Verification items for the finished model (mm, model axes). A direction names the side the tool comes from. Give positions to 0.01 mm unless a question says otherwise; leave off trailing zeros. Loops run counter-clockwise (first coordinate to the right, second up) from the corner with the lowest first, then second, coordinate; pieces in that order, holes last. Notation, with made-up numbers: M 36,28.25 L 46,28.25 A22 ccw 46,54.25 Z; hole C 35,87.5 d2. An arc over 180 degrees is marked long. Answer in a Markdown table with one row per item.
```python
from build123d import *

# Parameters (mm, degrees)
SKETCH1_W              = 10
SKETCH1_H              = 20
BOSS_EXTRUDE1_DEPTH    = 5
SKETCH2_W              = 10
SKETCH2_H              = 5
BOSS_EXTRUDE2_DEPTH    = 16
M2_5_CLEARANCE_HOLE1_D = 2.9
SKETCH6_W              = 10
SKETCH6_H              = 12
BOSS_EXTRUDE4_DEPTH    = 7
CHAMFER1_SIZE          = 3
CHAMFER1_SIZE2         = 5.196152423
FILLET1_R              = 4
CHAMFER2_SIZE          = 0.5
BOSS_EXTRUDE6_DEPTH    = 8
FILLET3_R              = 1
CHAMFER3_SIZE          = 0.5
CHAMFER3_SIZE2         = 2.83564091
SKETCH9_R              = 2
CUT_EXTRUDE1_DEPTH     = 2.1


with BuildPart() as part:
    # Sketch1 → Boss-Extrude1 (new body)
    with BuildSketch(Plane(origin=(0, 0, 0), x_dir=(1, 0, 0), z_dir=(0, 1, 0))):
        Rectangle(SKETCH1_W, SKETCH1_H)
    extrude(amount=BOSS_EXTRUDE1_DEPTH)

    # Sketch2 → Boss-Extrude2 (add)
    with BuildSketch(Plane(origin=(0, 0, 0), x_dir=(-1, 0, 0), z_dir=(0, -1, 0))):
        with Locations((0, 7.5)):
            Rectangle(SKETCH2_W, SKETCH2_H)
    extrude(amount=BOSS_EXTRUDE2_DEPTH)

    # M2.5 Clearance Hole1 (through all)
    with Locations(Plane.XY.offset(-5)):
        with Locations((0, -11.65), (0, -3.65)):
            Hole(M2_5_CLEARANCE_HOLE1_D / 2)

    # Sketch6 → Boss-Extrude4 (add)
    with BuildSketch(Plane.XY.offset(10)):
        with Locations((0, -1)):
            Rectangle(SKETCH6_W, SKETCH6_H)
    extrude(amount=BOSS_EXTRUDE4_DEPTH)

    # Chamfer1
    chamfer1_edges = [part.edges().sort_by_distance(p)[0] for p in [
        (0, 5, 17),
    ]]
    chamfer1_side = [part.faces().sort_by_distance(p)[0] for p in [
        (0, 5, 3.5),
    ]]
    chamfer(chamfer1_edges, length=CHAMFER1_SIZE, length2=CHAMFER1_SIZE2, reference=chamfer1_side[0])

    # Fillet1
    fillet1_edges = [part.edges().sort_by_distance(p)[0] for p in [
        (5, -7, 13.5),
        (-5, -7, 13.5),
    ]]
    fillet(fillet1_edges, radius=FILLET1_R)

    # Chamfer2
    chamfer2_edges = [part.edges().sort_by_distance(p)[0] for p in [
        (5, -16, -7.5),
        (-5, -16, -7.5),
    ]]
    chamfer(chamfer2_edges, length=CHAMFER2_SIZE)

    # Sketch8 → Boss-Extrude6 (add)
    with BuildSketch(Plane.XY.offset(17)):
        with BuildLine():
            ThreePointArc((-2.5, -4.5), (0, -7), (2.5, -4.5))
            ThreePointArc((2.5, -4.5), (0, -3.084524053), (-2.5, -4.5))
        make_face()
    extrude(amount=BOSS_EXTRUDE6_DEPTH)

    # Fillet3
    fillet3_edges = [part.edges().sort_by_distance(p)[0] for p in [
        (2.5, -4.5, 21),
        (-2.5, -4.5, 21),
    ]]
    fillet(fillet3_edges, radius=FILLET3_R)

    # Chamfer3
    chamfer3_edges = [part.edges().sort_by_distance(p)[0] for p in [
        (0, -3.084524053, 25),
        (0, -7, 25),
        (-2.442268543, -4.526279661, 25),
        (2.442268543, -4.526279661, 25),
    ]]
    chamfer3_side = [part.faces().sort_by_distance(p)[0] for p in [
        (0, -5.00792315, 25),
    ]]
    chamfer(chamfer3_edges, length=CHAMFER3_SIZE, length2=CHAMFER3_SIZE2, reference=chamfer3_side[0])

    # Sketch9 → Cut-Extrude1 (cut)
    with BuildSketch(Plane(origin=(0, 0, -10), x_dir=(-1, 0, 0), z_dir=(0, 0, -1))):
        with Locations((0, -3.65)):
            Circle(SKETCH9_R)
        with Locations((0, -11.65)):
            Circle(SKETCH9_R)
    extrude(amount=-CUT_EXTRUDE1_DEPTH, mode=Mode.SUBTRACT)


solid = part.part
```
Item 1: Release check for a two-part mould opening along X. For faces 6 (the cylindrical face through (-3.859, -5.797, 13.549)), 7 (the flat face through (-0.1, -2.8, 17)), 8 (the flat face through (0, -10, -7.9)) record: released by +X, released by -X, zero draft, split by the parting line, or undercut.
Reported:
| item | result |
|---|---|
| face 6 | released by -X |
| face 7 | zero draft |
| face 8 | undercut |
Item 2: Sectioned sample at D-D (x = 3.5). Record the cut outline in (y, z).
Reported:
| item | result |
|---|---|
| outline | M -16,-10 L 5,-10 L 5,14 L -0.2,17 L -6.12,17 L -6.12,10 L 0,10 L 0,-5 L -16,-5 Z |
Item 3: Sectioned sample at B-B (z = -6). Record the cut outline in (x, y), and give its area (3 significant figures).
Reported:
| item | result |
|---|---|
| outline | M -5,-15.5 L -4.5,-16 L 4.5,-16 L 5,-15.5 L 5,5 L -5,5 Z; hole C 0,-11.65 d2.9; hole C 0,-3.65 d2.9 |
| area | 197 mm^2 |
Item 4: Tool access check on faces 1 (the cylindrical face through (0.036, -3.085, 19.546)), 2 (the cylindrical face through (3.797, -5.859, 13.549)), 3 (the cylindrical face through (0.26, -9.667, -8.965)), 4 (the cylindrical face through (0, -7, 20)), 5 (the flat face through (0, -3, 10)). Record the directions out of +Z, -Z, +X, -X, +Y, -Y that give a thin tool (end or side, any length) a straight path to the whole face; none if there is none.
Reported:
| item | result |
|---|---|
| face 1 | +Z, +Y |
| face 2 | +Z, +X, -Y |
| face 3 | -Z |
| face 4 | +Z, -Y |
| face 5 | +X, -X, -Y |
Item 5: Go/stop test with flat-tipped pins: pin 1 (1 mm diameter, centred on x = 0, z = 12.5, fed in from -Y); pin 2 (3 mm diameter, centred on x = -1.5, z = 0.5, fed in from -Y); pin 3 (3.5 mm diameter, centred on x = 0, y = -11.65, fed in from -Z). Record where each tip stops, or that it passes through.
Reported:
| item | result |
|---|---|
| pin 1 | stops at y = -7 |
| pin 2 | stops at y = 0 |
| pin 3 | stops at z = -7.9 |
Item 6: Sectioned sample at A-A (y = -11.65). Record the cut outline in (x, z).
Reported:
| item | result |
|---|---|
| outline | M -5,-10 L -2,-10 L -2,-7.9 L -1.45,-7.9 L -1.45,-5 L -5,-5 Z; M 1.45,-7.9 L 2,-7.9 L 2,-10 L 5,-10 L 5,-5 L 1.45,-5 Z |
Item 7: Scan lines: L1, parallel to Y at x = 0, z = -9.35; L2, parallel to Y at x = 0, z = -5.55; L3, parallel to Z at x = 3, y = -0.25. Record each from-to range of solid material in increasing order. Write a range as [from, to].
Reported:
| item | result |
|---|---|
| L1 | y = [-16, -13.65], [-9.65, -5.65], [-1.65, 5] |
| L2 | y = [-16, -13.1], [-10.2, -5.1], [-2.2, 5] |
| L3 | z = [-10, -5], [10, 17] |
Item 8: Sectioned sample at C-C (z = 1). Record the cut outline in (x, y).
Reported:
| item | result |
|---|---|
| outline | M -5,0 L 5,0 L 5,5 L -5,5 Z |
